from build123d import *

# Parameters (mm, degrees)
UPRIGHT_PLATE_DEPTH          = 5
BASE_LUG_DEPTH               = 10
BASE_LUG_HOLE_PROFILE_R      = 10
BASE_LUG_HOLE_20_DEPTH       = 93.330926563
UPRIGHT_PLATE_HOLE_PROFILE_R = 10
UPRIGHT_PLATE_HOLE_20_DEPTH  = 95.868329805


with BuildPart() as part:
    # Upright Plate Profile → Upright Plate (new, symmetric)
    with BuildSketch(Plane.XY):
        with BuildLine():
            Line((0, 50), (30, 50))
            Line((30, 50), (70, 10))
            Line((70, 10), (70, 0))
            Line((70, 0), (0, 0))
            Line((0, 0), (0, 10))
            ThreePointArc((0, 10), (-20, 30), (0, 50))
        make_face()
    extrude(amount=UPRIGHT_PLATE_DEPTH, both=True)

    # Base Lug Profile → Base Lug (add)
    with BuildSketch(Plane.XZ):
        with BuildLine():
            Line((0, 5), (0, 25))
            ThreePointArc((0, 25), (20, 45), (40, 25))
            Line((40, 25), (40, 5))
            Line((40, 5), (70, 5))
            Line((70, 5), (70, -5))
            Line((70, -5), (0, -5))
            Line((0, -5), (0, 5))
        make_face()
    extrude(amount=-BASE_LUG_DEPTH)

    # Base Lug Hole Profile → Base Lug Hole Ø20 (cut, through all)
    with BuildSketch(Plane(origin=(0, 10, 0), x_dir=(1, 0, 0), z_dir=(0, 1, 0))):
        with Locations(Location((20, -25, 0), (0, 0, 270))):
            Circle(BASE_LUG_HOLE_PROFILE_R)
    extrude(amount=-BASE_LUG_HOLE_20_DEPTH, mode=Mode.SUBTRACT)

    # Upright Plate Hole Profile → Upright Plate Hole Ø20 (cut, through all)
    with BuildSketch(Plane.XY.offset(5)):
        with Locations((0, 30)):
            Circle(UPRIGHT_PLATE_HOLE_PROFILE_R)
    extrude(amount=-UPRIGHT_PLATE_HOLE_20_DEPTH, mode=Mode.SUBTRACT)


solid = part.part
Can you work these out from the model? Positions are in its coordinate system, mm. A direction names the side the tool comes from. Give positions to 0.01 mm unless a question says otherwise; leave off trailing zeros. Order: outer loops, then holes, each group sorted by start corner. A loop starts at its lowest first (then second) coordinate and runs counter-clockwise, first axis right, second up. Notation, with made-up numbers: (50.25, 49) - (61.25, 49) arc R28 ccw to (61.25, 78) - close; hole circle Ø9 at (88, -21). An arc over 180 degrees is marked (long way). Write each question's results on one line, items separated by ' | '.
1) Suppose I cut it at C-C, the plane y = 27. Write out the boundary of the cut face in (x, z).
Final values:
outline: (-19.77, -5) - (-9.54, -5) - (-9.54, 5) - (-19.77, 5) - close; (9.54, -5) - (53, -5) - (53, 5) - (9.54, 5) - close
2) Suppose I cut it at A-A, the plane x = 20. Write out the boundary of the cut face in (y, z).
Final values:
outline: (0, -5) - (50, -5) - (50, 5) - (10, 5) - (10, 15) - (0, 15) - close; (0, 35) - (10, 35) - (10, 45) - (0, 45) - close
3) I'm going to push flat-ended pins straight in: pin 1 Ø3 at (x, z) = (22, 34.5) entering from -Y; pin 2 Ø1.5 at (y, z) = (10.5, 35.5) entering from -X; pin 3 Ø12 at (x, z) = (14.5, 25.5) entering from +Y; pin 4 Ø5 at (y, z) = (2.5, 11) entering from +X. Where does each tip first touch, or does it pass through?
Final values:
pin 1: stops at y = 0 | pin 2: stops at x = 2.65 | pin 3: stops at y = 10 | pin 4: stops at x = 40
4) Please list where these lines run through material, in increasing order: line 1 along X through (y, z) = (4.5, 25); line 2 along Y through (x, z) = (29.5, 19); line 3 along X through (y, z) = (35, 3). Write a range as [from, to].
Final values:
line 1: x = [0, 10], [30, 40] | line 2: y = [0, 10] | line 3: x = [-19.36, -8.66], [8.66, 45]
5) If we mould it in two halves opening along X, with no side actions, what happens to faces 5 (the face through (23, 5.07, 34.54)), 6 (the face through (15, 50, 0)), 7 (the face through (-20, 30, 0))? For each: pulls with the +X half, pulls with the -X half, needs draft (parallel to the pull), parting line crosses it, or undercut.
Final values:
face 5: undercut | face 6: needs draft | face 7: pulls with the -X half
6) Suppose I cut it at D-D, the plane z = 3. Write out the boundary of the cut face in (x, y), then the cut area to 3 significant figures.
Final values:
outline: (0, 0) - (70, 0) - (70, 10) - (30, 50) - (0, 50) arc R20 ccw to (0, 10) - close; hole circle Ø20 at (0, 30) | area: 3,010 mm^2
7) On a 3-axis mill with a long thin cutter (end or side, diameter ignored), from which of +Z, -Z, +X, -X, +Y, -Y can I reach the whole of each face in a straight line? I mean faces 1 (the face through (0, 5, 10)), 2 (the face through (20, 10, 12)), 3 (the face through (40, 5, 15)), 4 (the face through (70, 5, 0)). Say none if no direction works.
Final values:
face 1: +Z, -Z, -X, -Y | face 2: +Z, +X, -X, +Y | face 3: +Z, +X, +Y, -Y | face 4: +Z, -Z, +X, +Y, -Y
8) Suppose I cut it at B-B, the plane z = 19. Write out the boundary of the cut face in (x, y).
Final values:
outline: (0, 0) - (12, 0) - (12, 10) - (0, 10) - close; (28, 0) - (40, 0) - (40, 10) - (28, 10) - close
